from build123d import *

# Parameters (mm, degrees)
SKETCH_1_W                   = 50
SKETCH_1_H                   = 25
EXTRUDE_1_DEPTH              = 15
CHAMFER_1_SIZE               = 2
HOLE_WIZARD_M5_1_D           = 5.5
HOLE_WIZARD_M5_1_CBORE_D     = 10
HOLE_WIZARD_M5_1_CBORE_DEPTH = 15.7


with BuildPart() as part:
    # 草图1 → 凸台-拉伸1 (new body)
    with BuildSketch(Plane.XY):
        Rectangle(SKETCH_1_W, SKETCH_1_H)
    extrude(amount=EXTRUDE_1_DEPTH)

    # 倒角1
    chamfer_1_edges = [part.edges().sort_by_distance(p)[0] for p in [
        (25, -12.5, 7.5),
        (-25, -12.5, 7.5),
    ]]
    chamfer(chamfer_1_edges, length=CHAMFER_1_SIZE)

    # M5 六角圆柱头螺钉的柱形沉头孔1 (through all)
    with Locations(Plane(origin=(0, -12.5, 0), x_dir=(-1, 0, 0), z_dir=(0, -1, 0))):
        with Locations((-17.5, -7.5), (17.5, -7.5)):
            CounterBoreHole(HOLE_WIZARD_M5_1_D / 2, HOLE_WIZARD_M5_1_CBORE_D / 2, HOLE_WIZARD_M5_1_CBORE_DEPTH)


solid = part.part
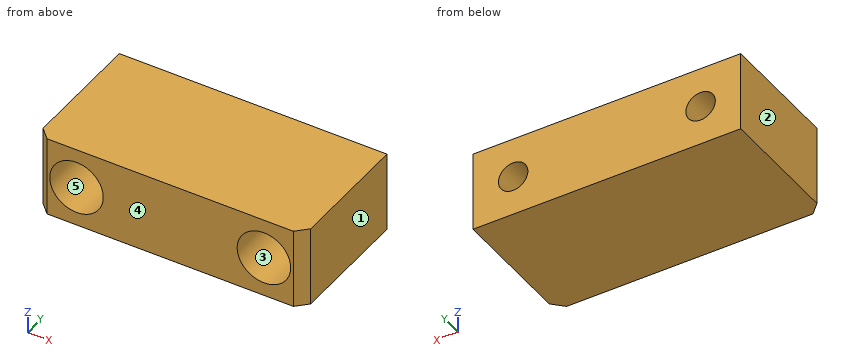
Verification items for the finished model (mm, model axes). Face numbers are marked on the shaded views. A direction names the side the tool comes from. Coordinates: 2 decimals unless noted, no trailing zeros. Order: outer loops, then holes, each group sorted by start corner. A loop starts at its lowest first (then second) coordinate and runs counter-clockwise, first axis right, second up. Notation, with made-up numbers: M 78.25,89 L 114.25,89 A25 ccw 114.25,117 Z; hole C 59,62 d1. An arc over 180 degrees is marked long. Return JSON: item names as keys, results as strings.
1) Gauge pin test, flat ends, axial feed: pin 1 (8 mm diameter, centred on x = -19.5, z = 7, fed in from -Y); pin 2 (8 mm diameter, centred on x = 17.5, z = 7.5, fed in from -Y). Record the tip position at first contact, or that the pin passes through.
Answer list:
{"pin 1": "y = -12.5", "pin 2": "y = 3.2"}
2) Cross-section at D-D, the plane z = 3.5. Record the boundary of the cut face in (x, y), and give its area (3 significant figures).
Answer list:
{"outline": "M -25,-10.5 L -23,-12.5 L -20.5,-12.5 L -20.5,3.2 L -14.5,3.2 L -14.5,-12.5 L 14.5,-12.5 L 14.5,3.2 L 20.5,3.2 L 20.5,-12.5 L 23,-12.5 L 25,-10.5 L 25,12.5 L -25,12.5 Z", "area": "1,060 mm2"}
3) Cross-section at C-C, the plane y = -9. Record the boundary of the cut face in (x, z), and give its area (3 significant figures).
Answer list:
{"outline": "M -25,0 L 25,0 L 25,15 L -25,15 Z; hole C -17.5,7.5 d10; hole C 17.5,7.5 d10", "area": "593 mm2"}
4) Release check for a two-part mould opening along X. For the marked faces 1, 2 and 3 record: +X half, -X half, draft (parallel to the pull), parting line (faces both ways), or undercut.
Answer list:
{"face 1": "+X half", "face 2": "-X half", "face 3": "undercut"}
5) Cross-section at B-B, the plane x = 17.5. Record the boundary of the cut face in (y, z), and give its area (3 significant figures).
Answer list:
{"outline": "M -12.5,0 L 12.5,0 L 12.5,4.75 L 3.2,4.75 L 3.2,2.5 L -12.5,2.5 Z; M -12.5,12.5 L 3.2,12.5 L 3.2,10.25 L 12.5,10.25 L 12.5,15 L -12.5,15 Z", "area": "167 mm2"}
6) Thickness scan on L1, parallel to Z at x = -17.5, y = -6.5; L2, parallel to Z at x = 17.5, y = 10; L3, parallel to X at y = 5.5, z = 6.5. Record the ranges inside material, lowest first. Write a range as [from, to].
Answer list:
{"L1": "[0, 2.5], [12.5, 15]", "L2": "[0, 4.75], [10.25, 15]", "L3": "[-25, -20.06], [-14.94, 14.94], [20.06, 25]"}
7) Access from +Z, -Z, +X, -X, +Y, -Y to the whole of each face (thin tool, end or side, straight path). Record for the marked faces 4 and 5.
Answer list:
{"face 4": "+Z, -Z, +X, -X, -Y", "face 5": "-Y"}
8) Cross-section at A-A, the plane z = 7.5. Record the boundary of the cut face in (x, y), and give its area (3 significant figures).
Answer list:
{"outline": "M -25,-10.5 L -23,-12.5 L -22.5,-12.5 L -22.5,3.2 L -20.25,3.2 L -20.25,12.5 L -25,12.5 Z; M -14.75,3.2 L -12.5,3.2 L -12.5,-12.5 L 12.5,-12.5 L 12.5,3.2 L 14.75,3.2 L 14.75,12.5 L -14.75,12.5 Z; M 20.25,3.2 L 22.5,3.2 L 22.5,-12.5 L 23,-12.5 L 25,-10.5 L 25,12.5 L 20.25,12.5 Z", "area": "830 mm2"}
